For this review, take the finished solid that the model builds, in its own axes (mm). A direction names the side the tool comes from. Give positions to 0.01 mm unless a question says otherwise; leave off trailing zeros. Write each loop counter-clockwise with the first axis right and the second up, starting at its lowest first coordinate (ties: lowest second). Pieces come first, ordered by that corner, then holes. Notation, with made-up numbers: M 21.25,-16 L 60.25,-16 A11 ccw 60.25,-12 Z; hole C -32,49.5 d9. An arc over 180 degrees is marked long. Write item = value, one per line.
```python
from build123d import *

# Parameters (mm, degrees)
SKETCH_2_R           = 3
BOSS_EXTRUDE_1_DEPTH = 12
SKETCH_3_R           = 2
BOSS_EXTRUDE_2_DEPTH = 1
BOSS_EXTRUDE_START   = 1.5
SKETCH_4_R           = 2
BOSS_EXTRUDE_3_DEPTH = 1.5
SKETCH_5_R           = 1.25
CUT_EXTRUDE_1_DEPTH  = 6
SKETCH_6_R           = 1.5
CUT_EXTRUDE_2_DEPTH  = 2.5
CUT_EXTRUDE_3_DEPTH  = 6
CUT_EXTRUDE_START    = -0.43115
SKETCH_11_R          = 0.5
CUT_EXTRUDE_8_DEPTH  = 1.93115


with BuildPart() as part:
    # Sketch 2 → Boss-Extrude 1 (new body)
    with BuildSketch(Plane(origin=(0, 0, 0), x_dir=(1, 0, 0), z_dir=(0, 1, 0))):
        with Locations(Location((0, 0, 0), (0, 0, 270))):
            Circle(SKETCH_2_R)
    extrude(amount=BOSS_EXTRUDE_1_DEPTH)

    # Sketch 3 → Boss-Extrude 2 (add)
    with BuildSketch(Plane(origin=(0, 12, 0), x_dir=(1, 0, 0), z_dir=(0, 1, 0))):
        with Locations(Location((0, 0, 0), (0, 0, 270))):
            Circle(SKETCH_3_R)
    extrude(amount=BOSS_EXTRUDE_2_DEPTH)

    # Sketch 4 → Boss-Extrude 3 (add)
    with BuildSketch(Plane(origin=(0, 0, 0), x_dir=(-1, 0, 0), z_dir=(0, -1, 0)).offset(BOSS_EXTRUDE_START)):
        with Locations(Location((0, 0, 0), (0, 0, 270))):
            Circle(SKETCH_4_R)
    extrude(amount=-BOSS_EXTRUDE_3_DEPTH)

    # Sketch 5 → Cut-Extrude 1 (cut)
    with BuildSketch(Plane(origin=(0, 13, 0), x_dir=(1, 0, 0), z_dir=(0, 1, 0))):
        with Locations(Location((0, 0, 0), (0, 0, 270))):
            Circle(SKETCH_5_R)
    extrude(amount=-CUT_EXTRUDE_1_DEPTH, mode=Mode.SUBTRACT)

    # Sketch 6 → Cut-Extrude 2 (cut)
    with BuildSketch(Plane(origin=(0, 7, 0), x_dir=(1, 0, 0), z_dir=(0, 1, 0))):
        with Locations(Location((0, 0, 0), (0, 0, 270))):
            Circle(SKETCH_6_R)
    extrude(amount=-CUT_EXTRUDE_2_DEPTH, mode=Mode.SUBTRACT)

    # Sketch 7 → Cut-Extrude 3 (cut)
    with BuildSketch(Plane(origin=(0, -1.5, 0), x_dir=(-1, 0, 0), z_dir=(0, -1, 0))):
        Polygon((-0.97407891, 1.14068851), (-1.385866178, -0.57391196), (0.117566508, -1.495385608), (1.458526276, -0.350287172), (0.783852304, 1.27889623), align=None)
    extrude(amount=-CUT_EXTRUDE_3_DEPTH, mode=Mode.SUBTRACT)

    # Sketch 11 → Cut-Extrude 8 (cut)
    with BuildSketch(Plane(origin=(-0.783852304, 0, -1.27889623), x_dir=(-0.8525974863360001, 0, 0.5225682025281811), z_dir=(-0.5225682025281811, 0, -0.8525974863360001)).offset(CUT_EXTRUDE_START)):
        with Locations(Location((-0.093426493, 1.5893341, 0), (0, 0, 180))):
            Circle(SKETCH_11_R)
    extrude(amount=CUT_EXTRUDE_8_DEPTH, mode=Mode.SUBTRACT)


solid = part.part
```
1. We need section A-A, the plane y = 10.5. Write out the cut boundary in (x, z), then the cut area to 3 significant figures.
Responses:
outline = C 0,0 d6; hole C 0,0 d2.5
area = 23.4 mm2
2. For line 1 along X through (y, z) = (5.75, 0); line 2 along Z through (x, y) = (-0.25, 7.5); line 3 along X through (y, z) = (10.3, 0), list the stretches that pass through material, from the lowest coordinate up. Write a range as from..to.
Responses:
line_1 = -3..-1.5, 1.5..3
line_2 = -2.99..-1.22, 1.22..2.99
line_3 = -3..-1.25, 1.25..3
3. We need section C-C, the plane z = 0. Write out the cut boundary in (x, y).
Responses:
outline = M -3,0 L -2,0 L -2,-1.5 L -1.31,-1.5 L -1.31,4.5 L -1.5,4.5 L -1.5,7 L -1.25,7 L -1.25,13 L -2,13 L -2,12 L -3,12 Z; M 1.25,-1.5 L 2,-1.5 L 2,0 L 3,0 L 3,12 L 2,12 L 2,13 L 1.25,13 L 1.25,7 L 1.5,7 L 1.5,4.5 L 1.25,4.5 Z
4. The part is to be moulded in two halves that separate along X. For faces 6 (the face through (-1.952, 12.493, -0.434)), 7 (the face through (-1, -1.5, 1)), 8 (the face through (0.083, 1.458, -1.211)), say which applies: +X half, -X half, draft (parallel to the pull), parting line (faces both ways), or undercut.
Responses:
face_6 = parting line
face_7 = draft
face_8 = undercut
5. We need section B-B, the plane x = 1.75. Write out the cut boundary in (y, z), then the cut area to 3 significant figures.
Responses:
outline = M -1.5,-0.97 L 0,-0.97 L 0,-2.44 L 12,-2.44 L 12,-0.97 L 13,-0.97 L 13,0.97 L 12,0.97 L 12,2.44 L 0,2.44 L 0,0.97 L -1.5,0.97 Z
area = 63.3 mm2
6. Insertion check: P1, Ø1.5, axis at y = 1.5, z = 2, coming from the +X side; P2, Ø2, axis at x = -1.5, y = 3, coming from the +Z side. Each pin has a flat end and moves straight along its axis. Give the tip position at first contact, or say it passes through.
Responses:
P1 = 2.73
P2 = 2.96
7. Machinability: for faces 1 (the face through (0.45, 5.77, 1.43)), 2 (the face through (-1, 12, 2)), 3 (the face through (1, 13, 1)), 4 (the face through (2, -1, 0)), 5 (the face through (0.9, 5.92, 2.86)), which of the approach directions +Z, -Z, +X, -X, +Y, -Y give a long, thin tool a straight path to every point of the face, cutting with its end or side? Answer none if there is none.
Responses:
face_1 = none
face_2 = +Y
face_3 = +Z, -Z, +X, -X, +Y
face_4 = -Y
face_5 = +Y, -Y
8. We need section D-D, the plane y = 1.25. Write out the cut boundary in (x, z).
Responses:
outline = M -1.79,-2.4 L -0.91,-0.97 L -1.46,0.35 L -0.12,1.5 L 1.39,0.57 L 0.97,-1.14 L -0.22,-1.23 L -1.16,-2.77 A3 ccw long Z
